```python
from build123d import *

# Parameters (mm, degrees)
SKETCH_1_W                = 60
SKETCH_1_H                = 60
EXTRUDE_1_DEPTH           = 10
SKETCH_2_W                = 60
SKETCH_2_H                = 10
EXTRUDE_2_DEPTH           = 50
CHAMFER_1_SIZE            = 3
HOLE_WIZARD_1_D           = 5.5
HOLE_WIZARD_1_DEPTH       = 15
HOLE_WIZARD_1_CBORE_D     = 10
HOLE_WIZARD_1_CBORE_DEPTH = 5.7
HOLE_WIZARD_1_TIP         = 1.652366702
HOLE_WIZARD_2_D           = 3.4
HOLE_WIZARD_2_DEPTH       = 15
HOLE_WIZARD_2_CBORE_D     = 6
HOLE_WIZARD_2_CBORE_DEPTH = 3.4
HOLE_WIZARD_2_TIP         = 1.021463052


with BuildPart() as part:
    # 草图1 → 凸台-拉伸1 (new body)
    with BuildSketch(Plane(origin=(0, 0, 0), x_dir=(1, 0, 0), z_dir=(0, 1, 0))):
        Rectangle(SKETCH_1_W, SKETCH_1_H)
    extrude(amount=EXTRUDE_1_DEPTH)

    # 草图2 → 凸台-拉伸2 (add)
    with BuildSketch(Plane(origin=(0, 10, 0), x_dir=(1, 0, 0), z_dir=(0, 1, 0))):
        with Locations((0, -25)):
            Rectangle(SKETCH_2_W, SKETCH_2_H)
    extrude(amount=EXTRUDE_2_DEPTH)

    # 倒角1
    chamfer_1_edges = [part.edges().sort_by_distance(p)[0] for p in [
        (-30, 60, 25),
        (30, 60, 25),
        (-30, 5, -30),
        (30, 5, -30),
    ]]
    chamfer(chamfer_1_edges, length=CHAMFER_1_SIZE)

    # 打孔尺寸(%根据)内六角圆柱头螺钉的类型1
    with Locations(Plane(origin=(0, 10, 0), x_dir=(1, 0, 0), z_dir=(0, 1, 0))):
        with Locations((-15, 20), (15, 20), (-15, -5), (15, -5)):
            CounterBoreHole(HOLE_WIZARD_1_D / 2, HOLE_WIZARD_1_CBORE_D / 2, HOLE_WIZARD_1_CBORE_DEPTH, depth=HOLE_WIZARD_1_DEPTH)
            with Locations((0, 0, -(HOLE_WIZARD_1_DEPTH + HOLE_WIZARD_1_TIP / 2))):  # 118° drill point
                Cone(0, HOLE_WIZARD_1_D / 2, HOLE_WIZARD_1_TIP, mode=Mode.SUBTRACT)

    # 打孔尺寸(%根据)内六角圆柱头螺钉的类型2
    with Locations(Plane(origin=(0, 0, 20), x_dir=(-1, 0, 0), z_dir=(0, 0, -1))):
        with Locations((-16.2, 48.2), (14.8, 48.2), (-16.2, 18.2), (14.8, 18.2)):
            CounterBoreHole(HOLE_WIZARD_2_D / 2, HOLE_WIZARD_2_CBORE_D / 2, HOLE_WIZARD_2_CBORE_DEPTH, depth=HOLE_WIZARD_2_DEPTH)
            with Locations((0, 0, -(HOLE_WIZARD_2_DEPTH + HOLE_WIZARD_2_TIP / 2))):  # 118° drill point
                Cone(0, HOLE_WIZARD_2_D / 2, HOLE_WIZARD_2_TIP, mode=Mode.SUBTRACT)


solid = part.part
```
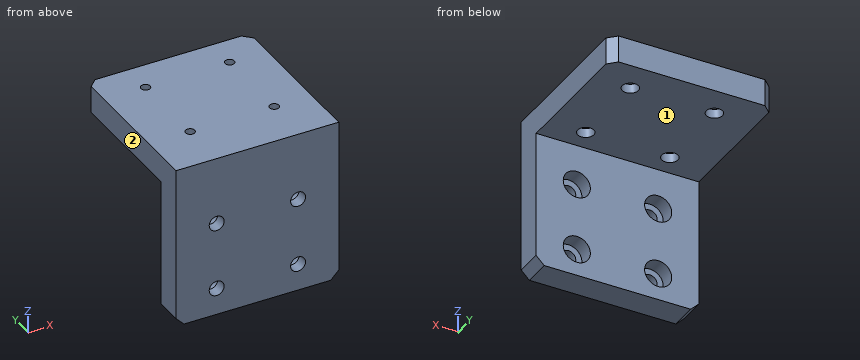
Geometry check sheet. Reference: the model listing, model coordinates, mm. Face numbers are marked on the shaded views. A direction names the side the tool comes from. Round coordinates to 2 decimals unless told otherwise and drop trailing zeros. Loops run counter-clockwise (first coordinate to the right, second up) from the corner with the lowest first, then second, coordinate; pieces in that order, holes last. Notation, with made-up numbers: (-17, 32.25) -> (-9, 32.25) arc R25 ccw to (-9, 57.25) -> close; hole circle Ø3 at (-11.75, -28). An arc over 180 degrees is marked (long way). Use a Markdown table: item, result.
(1) Sectioned sample at B-B (z = 22.5). Enter the section's corners in (x, y), then the cut area to 3 significant figures.
Calculated:
| item | result |
|---|---|
| outline | (-30, 0) -> (30, 0) -> (30, 57) -> (27, 60) -> (-27, 60) -> (-30, 57) -> close; hole circle Ø6 at (-14.8, 18.2); hole circle Ø6 at (-14.8, 48.2); hole circle Ø6 at (16.2, 18.2); hole circle Ø6 at (16.2, 48.2) |
| area | 3,480 mm² |
(2) Sectioned sample at C-C (x = -23). Enter the section's corners in (y, z).
Calculated:
| item | result |
|---|---|
| outline | (0, -30) -> (10, -30) -> (10, 20) -> (60, 20) -> (60, 30) -> (0, 30) -> close |
(3) Set-up check for the marked faces 1 and 2: record each of +Z, -Z, +X, -X, +Y, -Y from which the full face is reachable in a straight line by a thin tool's end or side.
Calculated:
| item | result |
|---|---|
| face 1 | -Z, +X, -X, +Y |
| face 2 | +Z, -Z, -X, +Y, -Y |
(4) Sectioned sample at D-D (y = 31). Enter the section's corners in (x, z), then the cut area to 3 significant figures.
Calculated:
| item | result |
|---|---|
| outline | (-30, 20) -> (30, 20) -> (30, 30) -> (-30, 30) -> close |
| area | 600 mm² |
(5) Sectioned sample at A-A (z = -20). Enter the section's corners in (x, y), then the cut area to 3 significant figures.
Calculated:
| item | result |
|---|---|
| outline | (-30, 0) -> (-17.75, 0) -> (-17.75, 4.3) -> (-20, 4.3) -> (-20, 10) -> (-30, 10) -> close; (-12.25, 0) -> (12.25, 0) -> (12.25, 4.3) -> (10, 4.3) -> (10, 10) -> (-10, 10) -> (-10, 4.3) -> (-12.25, 4.3) -> close; (17.75, 0) -> (30, 0) -> (30, 10) -> (20, 10) -> (20, 4.3) -> (17.75, 4.3) -> close |
| area | 439 mm² |
(6) Scan lines: probe 1 along Z at (x, y) = (-15, 6.5); probe 2 along Z at (x, y) = (-15, 2); probe 3 along X at (y, z) = (8.85, -20). Record each from-to range of solid material in increasing order.
Calculated:
| item | result |
|---|---|
| probe 1 | -30 to -25, -15 to 0, 10 to 30 |
| probe 2 | -30 to -22.75, -17.25 to 2.25, 7.75 to 30 |
| probe 3 | -30 to -20, -10 to 10, 20 to 30 |
(7) Go/stop test with flat-tipped pins: P1, Ø12, axis at x = -17.5, z = 12, coming from the +Y side; P2, Ø8, axis at x = 15, z = -20, coming from the +Y side; P3, Ø8, axis at x = -14.8, y = 18.2, coming from the -Z side. Record where each tip stops, or that it passes through.
Calculated:
| item | result |
|---|---|
| P1 | y = 10 |
| P2 | y = 4.3 |
| P3 | z = 20 |
